The model under review builds one solid part; all positions refer to its coordinate system, in mm. Face numbers are marked on the shaded views. A direction names the side the tool comes from. Give positions to 0.01 mm unless a question says otherwise; leave off trailing zeros. Loops run counter-clockwise (first coordinate to the right, second up) from the corner with the lowest first, then second, coordinate; pieces in that order, holes last. Notation, with made-up numbers: (32, 24) - (56, 24) arc R21 cw to (56, 57) - close; hole circle Ø7 at (-20, 34.5). An arc over 180 degrees is marked (long way). Answer as a JSON object with one key per item and string values.
from build123d import *

# Parameters (mm, degrees)
BASE_PLATE_SKETCH_R              = 5
BASE_PLATE_DEPTH                 = 15
CLEVIS_EAR_DEPTH                 = 8
CENTRE_CUT_DEPTH                 = 8
PIN_BORE_SKETCH_R                = 10
PIN_BORE_20_DEPTH                = 8
EAR_BOSS_SKETCH_W                = 50
EAR_BOSS_SKETCH_H                = 34
EAR_BOSS_DEPTH                   = 12
GUSSET_RIB_REACH                 = 92.967
GUSSET_SKETCH_WALL_W             = 207.257861566
GUSSET_SKETCH_WALL_H             = 6
COUNTERBORED_HOLE_16_D           = 16
COUNTERBORED_HOLE_16_DEPTH       = 49.839743178
COUNTERBORED_HOLE_16_CBORE_D     = 24
COUNTERBORED_HOLE_16_CBORE_DEPTH = 7


with BuildPart() as part:
    # Base Plate Sketch → Base Plate (new body)
    with BuildSketch(Plane(origin=(0, 0, 0), x_dir=(1, 0, 0), z_dir=(0, 1, 0))):
        with BuildLine():
            Line((-35, -25), (35, -25))
            ThreePointArc((35, -25), (42.071067812, -22.071067812), (45, -15))
            Line((45, -15), (45, 15))
            ThreePointArc((45, 15), (42.071067812, 22.071067812), (35, 25))
            Line((35, 25), (-35, 25))
            ThreePointArc((-35, 25), (-42.071067812, 22.071067812), (-45, 15))
            Line((-45, 15), (-45, -15))
            ThreePointArc((-45, -15), (-42.071067812, -22.071067812), (-35, -25))
        make_face()
        with Locations(Location((-35, 15, 0), (0, 0, 270))):
            Circle(BASE_PLATE_SKETCH_R, mode=Mode.SUBTRACT)
        with Locations(Location((35, 15, 0), (0, 0, 270))):
            Circle(BASE_PLATE_SKETCH_R, mode=Mode.SUBTRACT)
        with Locations(Location((-35, -15, 0), (0, 0, 270))):
            Circle(BASE_PLATE_SKETCH_R, mode=Mode.SUBTRACT)
        with Locations(Location((35, -15, 0), (0, 0, 270))):
            Circle(BASE_PLATE_SKETCH_R, mode=Mode.SUBTRACT)
    extrude(amount=BASE_PLATE_DEPTH)

    # Clevis Ear Sketch → Clevis Ear (add)
    with BuildSketch(Plane.XY.offset(25)):
        with BuildLine():
            Line((-25, 15), (-25, 50))
            ThreePointArc((-25, 50), (0, 75), (25, 50))
            Line((25, 50), (25, 15))
            Line((25, 15), (-25, 15))
        make_face()
    clevis_ear = extrude(amount=-CLEVIS_EAR_DEPTH)

    # Clevis Ear Mirror: Clevis Ear across plane
    add(clevis_ear.mirror(Plane.XY))

    # Centre Cut Sketch → Centre Cut (cut)
    with BuildSketch(Plane.XY.offset(25)):
        Polygon((-17.67766953, 50), (0, 67.67766953), (17.67766953, 50), (0, 32.32233047), align=None)
    extrude(amount=-CENTRE_CUT_DEPTH, mode=Mode.SUBTRACT)

    # Pin Bore Sketch → Pin Bore Ø20 (cut)
    with BuildSketch(Plane(origin=(0, 0, -25), x_dir=(-1, 0, 0), z_dir=(0, 0, -1))):
        with Locations((0, 50)):
            Circle(PIN_BORE_SKETCH_R)
    extrude(amount=-PIN_BORE_20_DEPTH, mode=Mode.SUBTRACT)

    # Ear Boss Sketch → Ear Boss (add)
    with BuildSketch(Plane(origin=(0, 15, 0), x_dir=(1, 0, 0), z_dir=(0, 1, 0))):
        Rectangle(EAR_BOSS_SKETCH_W, EAR_BOSS_SKETCH_H)
    extrude(amount=EAR_BOSS_DEPTH)

    # Gusset Sketch wall → Gusset Rib (add, up to next)
    with BuildSketch(Plane(origin=(35, 21, 0), x_dir=(0.857492925713, -0.514495755428, 0), z_dir=(0.514495755428, 0.857492925713, 0)), mode=Mode.PRIVATE) as gusset_rib_sk1:
        Rectangle(GUSSET_SKETCH_WALL_W, GUSSET_SKETCH_WALL_H)
    gusset_rib_tool1 = extrude(gusset_rib_sk1.sketch, amount=-GUSSET_RIB_REACH, mode=Mode.PRIVATE) - part.part
    gusset_rib = gusset_rib_tool1.solids().sort_by_distance((35, 21, 0))[0]
    add(gusset_rib)

    # Gusset Rib Mirror: Gusset Rib across plane
    add(gusset_rib.mirror(Plane(origin=(0, 0, 0), x_dir=(0, 0, 1), z_dir=(1, 0, 0))))

    # Counterbored Hole Ø16
    with Locations(Plane.ZX.offset(27)):
        with Locations((0, 0)):
            CounterBoreHole(COUNTERBORED_HOLE_16_D / 2, COUNTERBORED_HOLE_16_CBORE_D / 2, COUNTERBORED_HOLE_16_CBORE_DEPTH, depth=COUNTERBORED_HOLE_16_DEPTH)


solid = part.part
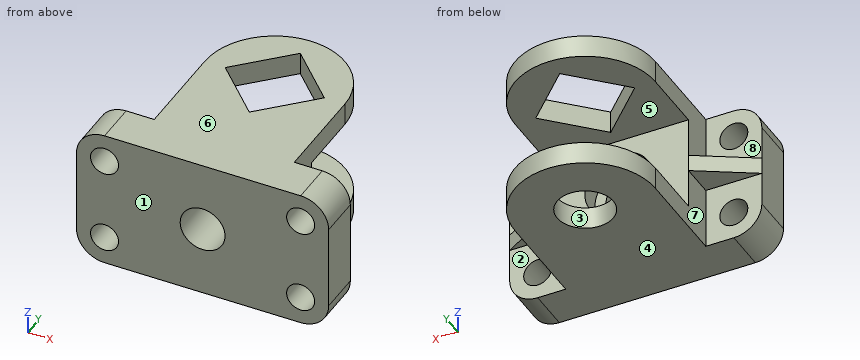
Q1. Consider section D-D, the plane y = 44.5. State the section outline as (x, z) points.
Results:
{"outline": "(-25, -25) - (-8.35, -25) - (-8.35, -17) - (-25, -17) - close; (-25, 17) - (-12.18, 17) - (-12.18, 25) - (-25, 25) - close; (8.35, -25) - (25, -25) - (25, -17) - (8.35, -17) - close; (12.18, 17) - (25, 17) - (25, 25) - (12.18, 25) - close"}
Q2. Consider section C-C, the plane y = 35.5. State the section outline as (x, z) points.
Results:
{"outline": "(-25, -25) - (25, -25) - (25, -17) - (-25, -17) - close; (-25, 17) - (-3.18, 17) - (-3.18, 25) - (-25, 25) - close; (3.18, 17) - (25, 17) - (25, 25) - (3.18, 25) - close"}
Q3. Consider section B-B, the plane z = 0. State the section outline as (x, y) points.
Results:
{"outline": "(-45, 0) - (-8, 0) - (-8, 20) - (-12, 20) - (-12, 27) - (-25, 27) - (-45, 15) - close; (8, 0) - (45, 0) - (45, 15) - (25, 27) - (12, 27) - (12, 20) - (8, 20) - close"}
Q4. For the marked faces 5, 6, 7 and 8, list the 3-axis set-ups (+Z, -Z, +X, -X, +Y, -Y) from which the entire face can be reached by the end or side of a thin tool; tool diameter is ignored.
Results:
{"face 5": "+X, -X, +Y", "face 6": "+Z, +X, -X, +Y, -Y", "face 7": "-Z, -X, +Y", "face 8": "+Z, -X, +Y"}
Q5. To check wall thickness, follow probe 1 along X at (y, z) = (5, -15); probe 2 along Z at (x, y) = (18, 59.5); probe 3 along X at (y, z) = (5, 0). State the ranges of each line that lie inside material, in increasing order. Write a range as [from, to].
Results:
{"probe 1": "x = [-45, -40], [-30, 30], [40, 45]", "probe 2": "z = [-25, -17], [17, 25]", "probe 3": "x = [-45, -8], [8, 45]"}
Q6. The part is to be moulded in two halves that separate along Y. For the marked faces 1, 2, 3 and 4, say which applies: +Y half, -Y half, draft (parallel to the pull), parting line (faces both ways), or undercut.
Results:
{"face 1": "-Y half", "face 2": "+Y half", "face 3": "undercut", "face 4": "draft"}
Q7. Consider section A-A, the plane z = 18.5. State the section outline as (x, y) points, plus the area to 3 significant figures.
Results:
{"outline": "(-44.37, 0) - (-38.57, 0) - (-38.57, 15) - (-44.37, 15) - close; (-31.43, 0) - (31.43, 0) - (31.43, 15) - (25, 15) - (25, 50) arc R25 ccw to (-25, 50) - (-25, 15) - (-31.43, 15) - close; (38.57, 0) - (44.37, 0) - (44.37, 15) - (38.57, 15) - close; hole (-17.68, 50) - (0, 32.32) - (17.68, 50) - (0, 67.68) - close", "area": "3,220 mm^2"}
Q8. Clearance check with flat-ended pins moving along their axes: pin 1 Ø6.5 at (y, z) = (39.5, -18) entering from +X; pin 2 Ø6 at (x, y) = (31, 19.5) entering from -Z; pin 3 Ø16 at (x, z) = (-35.5, 18) entering from +Y. State where each tip first meets the part, or that it passes through.
Results:
{"pin 1": "stops at x = 25", "pin 2": "stops at z = -3", "pin 3": "stops at y = 15"}
